Print and shaded views of the part. All mm, measured from the part's lowest x, y and z. A direction names the side the tool comes from. Round coordinates to 2 decimals unless told otherwise and drop trailing zeros. Loops run counter-clockwise (first coordinate to the right, second up) from the corner with the lowest first, then second, coordinate; pieces in that order, holes last. Notation, with made-up numbers: (-26.5, 43) - (23.5, 43) arc R29 ccw to (23.5, 75) - close; hole circle Ø6 at (60, 65.5). An arc over 180 degrees is marked (long way). Use one line per item in the form item = value. Start each with the question number.
Q1. Saw through at A-A (x = 7.5). Give the cut face in (y, z).
Q2. Pin check, flat tips, straight feed: pin 1 (3 mm diameter, centred on y = 8, z = 20.5, fed in from +X); pin 2 (1.5 mm diameter, centred on x = 10.5, z = 29, fed in from +Y); pin 3 (3 mm diameter, centred on x = 5, z = 6, fed in from -Y). Stop position of each tip, or through.
Q3. Drill centre lines: line 1 (Z direction, x = 7.5, y = 9.5); line 2 (Z direction, x = 9.25, y = 1); line 3 (X direction, y = 8.5, z = 42). Where is each one in solid material? Low to high.
Q4. 3-axis set-ups, long thin cutter, end or side, ignore diameter. For the marked faces 1 and 2: which of +Z, -Z, +X, -X, +Y, -Y reach the whole face in a straight line?
Q5. Saw through at B-B (z = 42). Give the cut face in (x, y), then the cut area to 3 significant figures.
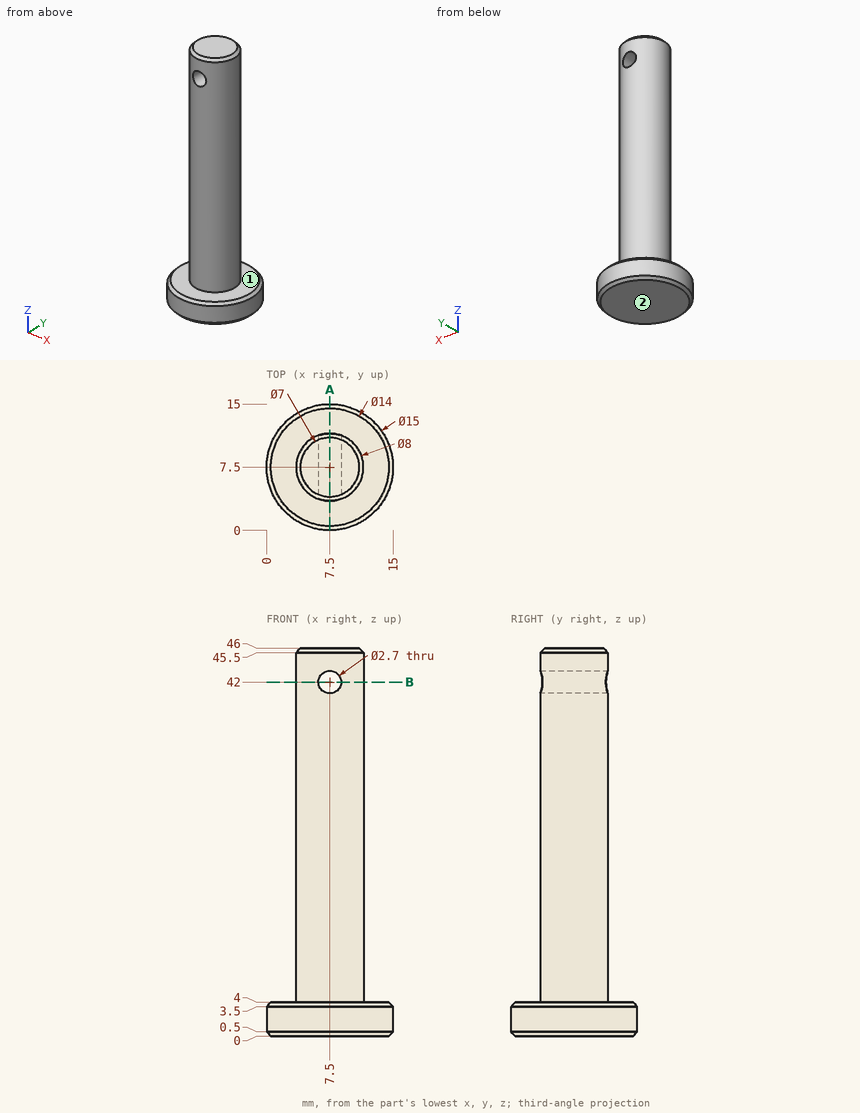
Report:
q1.outline = (0, 0.5) - (0.5, 0) - (14.5, 0) - (15, 0.5) - (15, 3.5) - (14.5, 4) - (11.5, 4) - (11.5, 40.65) - (3.5, 40.65) - (3.5, 4) - (0.5, 4) - (0, 3.5) - close; (3.5, 43.35) - (11.5, 43.35) - (11.5, 45.5) - (11, 46) - (4, 46) - (3.5, 45.5) - close
q2.pin_1 = 11.5
q2.pin_2 = 10.81
q2.pin_3 = 3.63
q3.line_1 = 0 to 40.65, 43.35 to 46
q3.line_2 = 0 to 4
q3.line_3 = 3.63 to 6.15, 8.85 to 11.37
q4.face_1 = +Z
q4.face_2 = -Z, +X, -X, +Y, -Y
q5.outline = (6.15, 3.73) - (6.15, 11.27) arc R4 ccw to start; (8.85, 3.73) arc R4 ccw to (8.85, 11.27) - close
q5.area = 29.1 mm²
